from build123d import *

# Parameters (mm, degrees)
EXTRUDE_1_DEPTH     = 1750
CUT_EXTRUDE_2_DEPTH = 100
CUT_REVOLVE_1_ANGLE = 90
EXTRUDE_2_DEPTH     = 1430


with BuildPart() as part:
    # 草图1 → 凸台-拉伸1 (new body)
    with BuildSketch(Plane.XY):
        with BuildLine():
            Line((-130, -144.49593989), (0, -144.49593989))
            Line((0, -144.49593989), (140, -144.49593989))
            Line((140, -144.49593989), (150.772266034, -162.999521413))
            Line((150.772266034, -162.999521413), (180.947633082, -162.999521413))
            Line((180.947633082, -162.999521413), (150.772266034, -104.49593989))
            Line((150.772266034, -104.49593989), (0, -104.49593989))
            Line((0, -104.49593989), (0, -4.49593989))
            Line((0, -4.49593989), (0, 75.50406011))
            Line((0, 75.50406011), (0, 185.50406011))
            Line((0, 185.50406011), (-107.776879674, 225.507843927))
            Line((-107.776879674, 225.507843927), (-185.49687967, 225.507843927))
            Line((-185.49687967, 225.507843927), (-185.49687967, 202.507843927))
            Line((-185.49687967, 202.507843927), (-99.70724302, 172.98245945))
            add(Edge.make_bspline(
                [(-99.70724302, 172.98245945), (-86.12473236, 169.546572985), (-80.854596401, 148.963344023), (-92.316673431, 140.10859264)],
                knots=[0, 0, 0, 0, 1, 1, 1, 1], degree=3))
            Line((-92.316673431, 140.10859264), (-152.70724302, 70.507843927))
            Line((-152.70724302, 70.507843927), (-179.70724302, 70.507843927))
            Line((-179.70724302, 70.507843927), (-179.70724302, 40.507843927))
            Line((-179.70724302, 40.507843927), (-152.70724302, 40.507843927))
            Line((-152.70724302, 40.507843927), (-102.0083923, -25.203763773))
            ThreePointArc((-102.0083923, -25.203763773), (-95.691769777, -48.530872609), (-107.72, -69.492156073))
            Line((-107.72, -69.492156073), (-185.49687967, -96.73098688))
            add(Edge.make_bspline(
                [(-187.99699364, -99.49593989), (-187.263883629, -97.683704139), (-185.49687967, -96.73098688)],
                knots=[0, 0, 0, 1, 1, 1], degree=2))
            Line((-187.99699364, -99.49593989), (-187.99699364, -129.49593989))
            Line((-187.99699364, -129.49593989), (-140.29956323, -129.49593989))
            Line((-140.29956323, -129.49593989), (-130, -144.49593989))
        make_face()
    extrude(amount=-EXTRUDE_1_DEPTH)

    # 草图2 → 切除-拉伸2 (cut)
    with BuildSketch(Plane.XY):
        with BuildLine():
            Line((0, 75.50406011), (0, -4.49593989))
            Line((0, -4.49593989), (-20, -4.49593989))
            ThreePointArc((-20, -4.49593989), (-60, 35.50406011), (-20, 75.50406011))
            Line((-20, 75.50406011), (0, 75.50406011))
        make_face()
    cut_extrude_2 = extrude(amount=-CUT_EXTRUDE_2_DEPTH, mode=Mode.SUBTRACT)

    # 草图4 → 切除-旋转1 (revolve, cut)
    with BuildSketch(Plane(origin=(0, 0, 0), x_dir=(0, 0, -1), z_dir=(1, 0, 0))):
        with BuildLine():
            Line((100, 95.50406011), (100, -24.49593989))
            ThreePointArc((100, -24.49593989), (160, 35.50406011), (100, 95.50406011))
        make_face()
    cut_revolve_1 = revolve(axis=Axis((0, 95.50406011, -100), (0, 1, 0)), revolution_arc=CUT_REVOLVE_1_ANGLE, mode=Mode.SUBTRACT)

    # 镜向1: 切除-拉伸2, 切除-旋转1 across plane
    add(cut_extrude_2.mirror(Plane.XY.offset(-875)), mode=Mode.SUBTRACT)
    add(cut_revolve_1.mirror(Plane.XY.offset(-875)), mode=Mode.SUBTRACT)

    # 草图6 → 凸台-拉伸2 (add)
    with BuildSketch(Plane.XY.offset(-160)):
        Polygon((0, 185.50406011), (63.207169624, 162.043314569), (103.142950665, 147.220262017), (103.142950665, -104.49593989), (83.175060144, -104.49593989), (83.175060144, 133.726046688), (0, 164.598318505), align=None)
    extrude(amount=-EXTRUDE_2_DEPTH)


solid = part.part
Geometry check sheet. Reference: the model listing, model coordinates, mm. A direction names the side the tool comes from. Coordinates: 2 decimals unless noted, no trailing zeros. Order: outer loops, then holes, each group sorted by start corner. A loop starts at its lowest first (then second) coordinate and runs counter-clockwise, first axis right, second up. Notation, with made-up numbers: (2.5, 55) - (52.5, 55) arc R17 ccw to (52.5, 79) - close; hole circle Ø3 at (76, -25.5). An arc over 180 degrees is marked (long way). Answer in a Markdown table with one row per item. Add a question column.
1) Gauge pin test, flat ends, axial feed: P1, Ø6, axis at x = -7, z = -44.5, coming from the +Y side; P2, Ø10, axis at x = -29.5, z = -430, coming from the +Y side; P3, Ø10, axis at y = 33, z = -1291.5, coming from the -X side. Record the tip position at first contact, or that the pin passes through.
2) Cross-section at A-A, the plane x = 37. Record the cut outline in (y, z).
3) Set-up check for faces 5 (the flat face through (-122.089, 105.795, -862.75)), 6 (the flat face through (3, -144.496, -863)), 7 (the cylindrical face through (-59.99, 34.62, -49.3)), 8 (the flat face through (83.175, 13, -865)), 9 (the cylindrical face through (-59.99, 34.62, -1700.7)): record each of +Z, -Z, +X, -X, +Y, -Y from which the full face is reachable in a straight line by a thin tool's end or side.
4) Release check for a two-part mould opening along X. For faces 1 (the flat face through (42.17, 148.946, -864.99)), 2 (the flat face through (166.071, -134.157, -862.75)), 3 (the flat face through (-164, -129.496, -863)), 4 (the flat face through (-143.2, 187.95, -862.75)) record: +X half, -X half, draft (parallel to the pull), parting line (faces both ways), or undercut.
5) Material ranges on line 1 along X through (y, z) = (126, -195); line 2 along Y through (x, z) = (-170, -291.5); line 3 along Y through (x, z) = (-105.5, -258), recorded low to high. Write a range as [from, to].
Check result:
| question | item | result |
|---|---|---|
| 1 | P1 | stops at y = 189.22 |
| 1 | P2 | stops at y = 198.31 |
| 1 | P3 | stops at x = -150.77 |
| 2 | outline | (-144.5, -1750) - (-104.5, -1750) - (-104.5, 0) - (-144.5, 0) - close; (150.86, -1590) - (171.77, -1590) - (171.77, -160) - (150.86, -160) - close |
| 3 | face 5 | +Z, -Z, -X |
| 3 | face 6 | +Z, -Z, -X, -Y |
| 3 | face 7 | +Z, +X |
| 3 | face 8 | +Z, -Z |
| 3 | face 9 | -Z, +X |
| 4 | face 1 | undercut |
| 4 | face 2 | +X half |
| 4 | face 3 | draft |
| 4 | face 4 | -X half |
| 5 | line 1 | x = [-104.56, 0], [83.18, 103.14] |
| 5 | line 2 | y = [-129.5, -91.3], [40.51, 70.51], [197.17, 225.51] |
| 5 | line 3 | y = [-144.5, -67.61], [-20.68, 124.91], [174.98, 224.66] |
